Verification items for the finished model (mm, model axes). A direction names the side the tool comes from. Round coordinates to 2 decimals unless told otherwise and drop trailing zeros. Order: outer loops, then holes, each group sorted by start corner. A loop starts at its lowest first (then second) coordinate and runs counter-clockwise, first axis right, second up. Notation, with made-up numbers: M -38,-3.5 L -3,-3.5 A29 ccw -3,20.5 Z; hole C 23.25,25.5 d7. An arc over 180 degrees is marked long. Write item = value, one per line. Start each with the question number.
from build123d import *

# Parameters (mm, degrees)
BRACKET_BODY_DEPTH      = 50
TOP_GROOVE_SKETCH_W     = 25
TOP_GROOVE_SKETCH_H     = 20
TOP_GROOVE_CUT_DEPTH    = 20
NOTCH_SKETCH_W          = 20
NOTCH_SKETCH_H          = 20
NOTCH_CUT_DEPTH         = 111.566721937
MOUNTING_HOLES_SKETCH_R = 6
MOUNTING_HOLES_2X_DEPTH = 128.279220614


with BuildPart() as part:
    # Bracket Profile Sketch → Bracket Body (new body)
    with BuildSketch(Plane.XY):
        with BuildLine():
            Line((0, 0), (65, 0))
            ThreePointArc((65, 0), (85, 20), (105, 0))
            Line((105, 0), (110, 0))
            Line((110, 0), (110, 50))
            Line((110, 50), (85, 50))
            Line((85, 50), (30, 20))
            Line((30, 20), (30, 10))
            Line((30, 10), (0, 10))
            Line((0, 10), (0, 0))
        make_face()
    extrude(amount=BRACKET_BODY_DEPTH)

    # Top Groove Sketch → Top Groove Cut (cut)
    with BuildSketch(Plane(origin=(0, 50, 0), x_dir=(1, 0, 0), z_dir=(0, 1, 0))):
        with Locations((97.5, -25)):
            Rectangle(TOP_GROOVE_SKETCH_W, TOP_GROOVE_SKETCH_H)
    extrude(amount=-TOP_GROOVE_CUT_DEPTH, mode=Mode.SUBTRACT)

    # Notch Sketch → Notch Cut (cut, through all)
    with BuildSketch(Plane(origin=(85, 0, 0), x_dir=(0, 0, -1), z_dir=(1, 0, 0))):
        with Locations((-25, 40)):
            Rectangle(NOTCH_SKETCH_W, NOTCH_SKETCH_H)
    extrude(amount=-NOTCH_CUT_DEPTH, mode=Mode.SUBTRACT)

    # Mounting Holes Sketch → Mounting Holes 2x (cut, through all)
    with BuildSketch(Plane(origin=(0, 10, 0), x_dir=(1, 0, 0), z_dir=(0, 1, 0))):
        with Locations(Location((15, -12, 0), (0, 0, 270))):
            Circle(MOUNTING_HOLES_SKETCH_R)
        with Locations(Location((15, -38, 0), (0, 0, 270))):
            Circle(MOUNTING_HOLES_SKETCH_R)
    extrude(amount=-MOUNTING_HOLES_2X_DEPTH, mode=Mode.SUBTRACT)


solid = part.part
1) Cross-section at D-D, the plane z = 28.5. Enter the section's corners in (x, y).
2) Access from +Z, -Z, +X, -X, +Y, -Y to the whole of each face (thin tool, end or side, straight path). Record for faces 1 (the flat face through (79, 30, 25)), 2 (the flat face through (15, 10, 25)), 3 (the flat face through (66, 20, 50)).
3) Scan lines: probe 1 along X at (y, z) = (3.75, 38); probe 2 along X at (y, z) = (7.75, 38); probe 3 along Z at (x, y) = (17, 5). Record each from-to range of solid material in increasing order.
4) Cross-section at C-C, the plane z = 12. Enter the section's corners in (x, y), then the cut area to 3 significant figures.
5) Cross-section at B-B, the plane y = 32. Enter the section's corners in (x, z), then the cut area to 3 significant figures.
6) Cross-section at A-A, the plane x = 15. Enter the section's corners in (y, z).
7) Gauge pin test, flat ends, axial feed: P1, Ø6, axis at x = 81, y = 17, coming from the +Z side; P2, Ø12, axis at x = 76.5, z = 35.5, coming from the +Y side; P3, Ø16, axis at x = 67, z = 28.5, coming from the +Y side; P4, Ø1.5, axis at x = 28.5, z = 11.5, coming from the +Y side. Record the tip position at first contact, or that the pin passes through.
8) Release check for a two-part mould opening along X. For faces 4 (the flat face through (98, 50, 7)), 5 (the flat face through (30, 15, 25)), 6 (the cylindrical face through (15, 5, 32)) record: pulls with the +X half, pulls with the -X half, needs draft (parallel to the pull), parting line crosses it, or undercut.
Geometry results:
q1.outline = M 0,0 L 65,0 A20 cw 105,0 L 110,0 L 110,30 L 48.33,30 L 30,20 L 30,10 L 0,10 Z
q2.face_1 = +X, -X, +Y
q2.face_2 = +Z, -Z, -X, +Y
q2.face_3 = +Z, +X, -X, +Y, -Y
q3.probe_1 = 0 to 9, 21 to 65.35, 104.65 to 110
q3.probe_2 = 0 to 9, 21 to 66.56, 103.44 to 110
q3.probe_3 = 0 to 6.34, 17.66 to 32.34, 43.66 to 50
q4.outline = M 0,0 L 9,0 L 9,10 L 0,10 Z; M 21,0 L 65,0 A20 cw 105,0 L 110,0 L 110,50 L 85,50 L 30,20 L 30,10 L 21,10 Z
q4.area = 2,730 mm^2
q5.outline = M 52,0 L 110,0 L 110,15 L 52,15 Z; M 52,35 L 110,35 L 110,50 L 52,50 Z
q5.area = 1,740 mm^2
q6.outline = M 0,0 L 10,0 L 10,6 L 0,6 Z; M 0,18 L 10,18 L 10,32 L 0,32 Z; M 0,44 L 10,44 L 10,50 L 0,50 Z
q7.P1 = 50
q7.P2 = 48.64
q7.P3 = 42.73
q7.P4 = 10
q8.face_4 = needs draft
q8.face_5 = pulls with the -X half
q8.face_6 = undercut
